Check sheet for the drawn part. Datum: minimum x, y, z corner. Units: mm. A direction names the side the tool comes from. Give positions to 0.01 mm unless a question says otherwise; leave off trailing zeros. Loops run counter-clockwise (first coordinate to the right, second up) from the corner with the lowest first, then second, coordinate; pieces in that order, holes last.
1. Tool access check on the marked faces 1 and 2. Record the directions out of +Z, -Z, +X, -X, +Y, -Y that give a thin tool (end or side, any length) a straight path to the whole face; none if there is none.
2. Cross-section at A-A, the plane z = 8. Record the cut outline in (x, y), plus the area to 3 significant figures.
3. Go/stop test with flat-tipped pins: pin 1 Ø5 at (x, y) = (10.5, 6.5) entering from -Z; pin 2 Ø6.5 at (y, z) = (8, 7) entering from -X; pin 3 Ø1 at (x, y) = (24, 8.5) entering from +Z; pin 4 Ø1.5 at (x, z) = (20.5, 11.5) entering from -Y. Record where each tip stops, or that it passes through.
4. Cross-section at C-C, the plane x = 28. Record the cut outline in (y, z), plus the area to 3 significant figures.
5. Cross-section at D-D, the plane y = 14.5. Record the cut outline in (x, z), plus the area to 3 significant figures.
6. Material ranges on L1, parallel to X at y = 1.75, z = 6; L2, parallel to Y at x = 10.5, z = 8.25; L3, parallel to Z at x = 16, y = 8, recorded low to high.
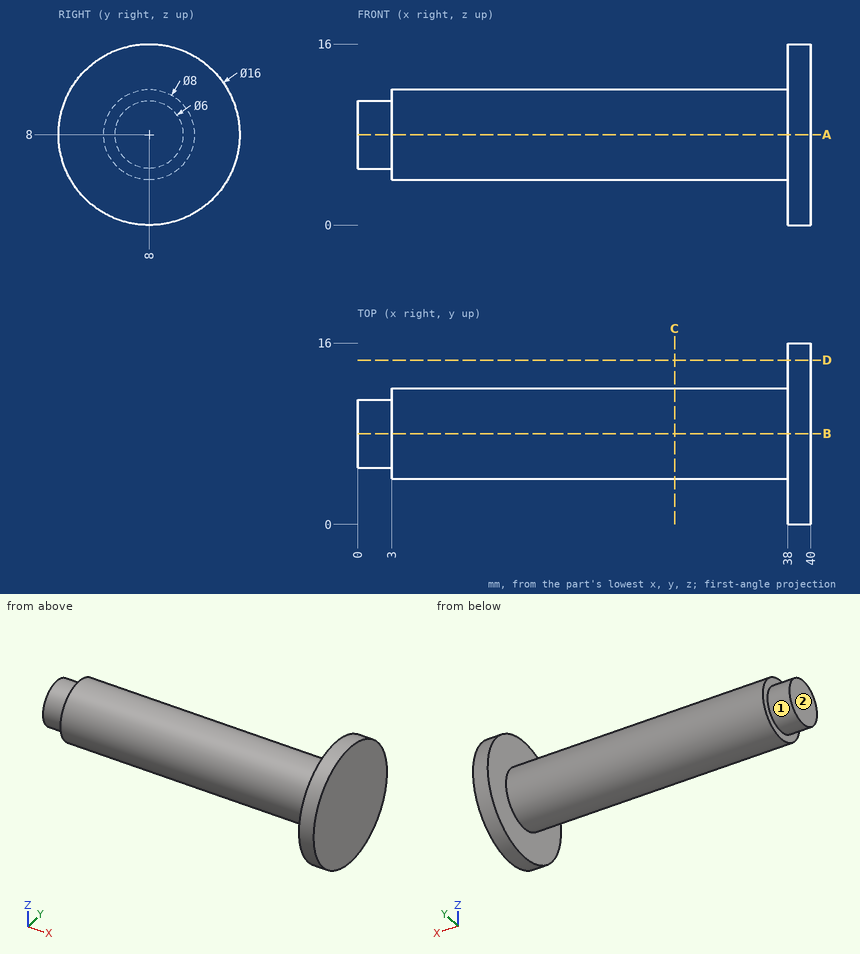
Result:
1. face 1: -X
1. face 2: +Z, -Z, -X, +Y, -Y
2. outline: (0, 5) - (3, 5) - (3, 4) - (38, 4) - (38, 0) - (40, 0) - (40, 16) - (38, 16) - (38, 12) - (3, 12) - (3, 11) - (0, 11) - close
2. area: 330 mm2
3. pin 1: stops at z = 4
3. pin 2: stops at x = 0
3. pin 3: stops at z = 12
3. pin 4: stops at y = 5.1
4. outline: circle Ø8 at (8, 8)
4. area: 50.3 mm2
5. outline: (38, 3.34) - (40, 3.34) - (40, 12.66) - (38, 12.66) - close
5. area: 18.7 mm2
6. L1: x = 38 to 40
6. L2: y = 4.01 to 11.99
6. L3: z = 4 to 12
